from build123d import *

# Parameters (mm, degrees)
SKETCH_3_R          = 4.889549894
CUT_EXTRUDE_1_DEPTH = 5


with BuildPart() as part:
    # 草图2 → 放样1 section 0
    with BuildSketch(Plane.XY.offset(-350)):
        with BuildLine():
            Line((-30, 25), (30, 25))
            Line((30, 25), (30, -25))
            Line((30, -25), (-30, -25))
            Line((-30, -25), (-30, 25))
        make_face()
    # 草图1 for 放样1 → 放样1 section 1
    with BuildSketch(Plane.XY):
        with BuildLine():
            # circular arc as an exact rational Bezier (weights 1, cos(half-angle), 1)
            Bezier((-11.523319194, 9.602765995), (0, 23.430749028), (11.523319194, 9.602765995), weights=[1, 0.6401844, 1])
            Bezier((11.523319194, 9.602765995), (19.52562419, 0), (11.523319194, -9.602765995), weights=[1, 0.76822128, 1])
            Bezier((11.523319194, -9.602765995), (0, -23.430749028), (-11.523319194, -9.602765995), weights=[1, 0.6401844, 1])
            Bezier((-11.523319194, -9.602765995), (-19.52562419, 0), (-11.523319194, 9.602765995), weights=[1, 0.76822128, 1])
        make_face()
    loft()

    # 草图3 → 切除-拉伸1 (cut)
    with BuildSketch(Plane.XY):
        Circle(SKETCH_3_R)
    extrude(amount=-CUT_EXTRUDE_1_DEPTH, mode=Mode.SUBTRACT)


solid = part.part
Verification items for the finished model (mm, model axes). Round coordinates to 2 decimals unless told otherwise and drop trailing zeros. Write each question's results on one line, items separated by ' | '.
1) Gauge pin test, flat ends, axial feed: P1, Ø8, axis at x = -15.5, z = -174.5, coming from the +Y side; P2, Ø5, axis at x = 0, y = -0.5, coming from the +Z side; P3, Ø1.5, axis at y = 12, z = -60.5, coming from the +X side. Record the tip position at first contact, or that the pin passes through.
Checks:
P1: stops at y = 19.12 | P2: stops at z = -5 | P3: stops at x = 15.19
2) Scan lines: L1, parallel to Y at x = 0, z = -1; L2, parallel to X at y = -11, z = -105; L3, parallel to X at y = 0.5, z = -135. Record each from-to range of solid material in increasing order. Write a range as from..to.
Checks:
L1: y = -15.03..-4.89, 4.89..15.03 | L2: x = -18.04..18.04 | L3: x = -20.78..20.78
3) Mould release check, pull along X, two halves, no side actions. Record for faces 1 (the flat face through (0, 6, 0)), 2 (the cylindrical face through (4.664, 1.469, -2.465)), 3 (the flat face through (0, 0, -5)): released by +X, released by -X, zero draft, split by the parting line, or undercut.
Checks:
face 1: zero draft | face 2: undercut | face 3: undercut
